Source: CAD feature listing. Evaluate the final solid. Frame: model axes, mm. Coordinates: 2 decimals unless noted, no trailing zeros. Write each loop counter-clockwise with the first axis right and the second up, starting at its lowest first coordinate (ties: lowest second). Pieces come first, ordered by that corner, then holes. Notation, with made-up numbers: (-36.75, -21.5) - (18.25, -21.5) arc R38 ccw to (18.25, 16.5) - close; hole circle Ø3 at (3, -0.5). An arc over 180 degrees is marked (long way). One line per question, with ' | ' between items. Start each with the question number.
Q1. Cut plane B-B, the plane x = 27.5. Return loops of the section in (y, z), plus the area to 3 significant figures.
Q2. Line query: line 1 (Y direction, x = -27.5, z = 1.7); line 2 (Y direction, x = -30.5, z = 1.3); line 3 (X direction, y = 27.5, z = 3.75). Output: solid intervals per line, ascending.
Q3. Cut plane A-A, the plane y = -29. Return loops of the section in (x, z), plus the area to 3 significant figures.
Q4. Contact query for flat-ended pins moving along their axis: P1, Ø7.5, axis at x = 27.5, y = -29, coming from the -Z side; P2, Ø1, axis at x = -1.5, y = -12.5, coming from the -Z side. Output: stop coordinate, or through.
Q5. Draft query along Y for faces 1 (the face through (-30.87, 26.41, 2.96)), 2 (the face through (-31.746, -28.813, 2.958)), 3 (the face through (1, 1, 0)), 4 (the face through (35, -35, 3)). Return one class per face: +Y half, -Y half, draft (parallel to the pull), parting line (faces both ways), or undercut.
Q6. Cut plane C-C, the plane z = 3.3. Return loops of the section in (x, y), plus the area to 3 significant figures.
```python
from build123d import *

# Parameters (mm, degrees)
SKETCH1_R           = 4.25
BOSS_EXTRUDE1_DEPTH = 6


with BuildPart() as part:
    # Sketch1 → Boss-Extrude1 (new body)
    with BuildSketch(Plane.XY):
        Polygon((-37.5, 32.5), (-32.5, 37.5), (32.5, 37.5), (37.5, 32.5), (37.5, -32.5), (32.5, -37.5), (-32.5, -37.5), (-37.5, -32.5), align=None)
        with Locations((-27.5, 29)):
            Circle(SKETCH1_R, mode=Mode.SUBTRACT)
        with Locations((27.5, 29)):
            Circle(SKETCH1_R, mode=Mode.SUBTRACT)
        with Locations((-27.5, -29)):
            Circle(SKETCH1_R, mode=Mode.SUBTRACT)
        with Locations((27.5, -29)):
            Circle(SKETCH1_R, mode=Mode.SUBTRACT)
    extrude(amount=BOSS_EXTRUDE1_DEPTH)


solid = part.part
```
Reply:
1) outline: (-37.5, 0) - (-33.25, 0) - (-33.25, 6) - (-37.5, 6) - close; (-24.75, 0) - (24.75, 0) - (24.75, 6) - (-24.75, 6) - close; (33.25, 0) - (37.5, 0) - (37.5, 6) - (33.25, 6) - close | area: 348 mm^2
2) line 1: y = -37.5 to -33.25, -24.75 to 24.75, 33.25 to 37.5 | line 2: y = -37.5 to -32.01, -25.99 to 25.99, 32.01 to 37.5 | line 3: x = -37.5 to -31.48, -23.52 to 23.52, 31.48 to 37.5
3) outline: (-37.5, 0) - (-31.75, 0) - (-31.75, 6) - (-37.5, 6) - close; (-23.25, 0) - (23.25, 0) - (23.25, 6) - (-23.25, 6) - close; (31.75, 0) - (37.5, 0) - (37.5, 6) - (31.75, 6) - close | area: 348 mm^2
4) P1: passes through | P2: stops at z = 0
5) face 1: undercut | face 2: undercut | face 3: draft | face 4: -Y half
6) outline: (-37.5, -32.5) - (-32.5, -37.5) - (32.5, -37.5) - (37.5, -32.5) - (37.5, 32.5) - (32.5, 37.5) - (-32.5, 37.5) - (-37.5, 32.5) - close; hole circle Ø8.5 at (-27.5, -29); hole circle Ø8.5 at (-27.5, 29); hole circle Ø8.5 at (27.5, -29); hole circle Ø8.5 at (27.5, 29) | area: 5,350 mm^2
